Geometry: final body of the model. Coordinates: model frame, mm. A direction names the side the tool comes from. Give positions to 0.01 mm unless a question says otherwise; leave off trailing zeros. Loops run counter-clockwise (first coordinate to the right, second up) from the corner with the lowest first, then second, coordinate; pieces in that order, holes last. Notation, with made-up numbers: (12, 47) -> (56, 47) arc R31 cw to (56, 77) -> close; hole circle Ø11 at (-38.5, 65.5). An arc over 180 degrees is marked (long way). Answer in a Markdown table with one row per item. Add a question column.
1) Section query A-A (x = 40). Return the cut outline in (y, z).
2) Section query D-D (x = 105). Return the cut outline in (y, z).
3) Access query for faces 1 (the flat face through (25, 10, 5)), 2 (the flat face through (40, 6.8, 56)), 3 (the cylindrical face through (-40.43, 9.44, 49.23)). Directions: +Z, -Z, +X, -X, +Y, -Y. A direction counts if a zero-diameter tool reaches every point of the face in a straight line with its end or side. Return the directions, or none.
4) Section query C-C (z = -45). Return the cut outline in (x, y).
5) Line query: line 1 (X direction, y = 10.25, z = -45); line 2 (Z direction, x = -105, y = 10); line 3 (X direction, y = 10.6, z = 52.5). Output: solid intervals per line, ascending. Write a range as from..to.
6) First-contact query: P1, Ø3.5, axis at x = -103, z = -46, coming from the -Y side; P2, Ø3, axis at x = -24, z = 5, coming from the +Y side; P3, Ø6, axis at x = -105, z = 45, coming from the +Y side. Flat tips, straight axial feed; report the tip coordinate or a pass-through.
7) Draft query along Z for faces 4 (the cylindrical face through (110.495, 3.352, 44.758)), 5 (the flat face through (-2, 6, 72.5)), 6 (the flat face through (-2, 12, -1)). Return one class per face: +Z half, -Z half, draft (parallel to the pull), parting line (faces both ways), or undercut.
8) Section query B-B (z = -20). Return the cut outline in (x, y), plus the area to 3 significant figures.
```python
from build123d import *

# Parameters (mm, degrees)
SKETCH_1_W                   = 250
SKETCH_1_H                   = 145
EXTRUDE_1_DEPTH              = 12
CHAMFER_1_SIZE               = 2
SKETCH_2_R                   = 18
CUT_EXTRUDE_1_DEPTH          = 146.000862066
HOLE_WIZARD_M4_1_D           = 3.3
HOLE_WIZARD_M6_1_D           = 6.6
HOLE_WIZARD_M6_1_CBORE_D     = 11
HOLE_WIZARD_M6_1_CBORE_DEPTH = 6.8
SKETCH_11_R                  = 5
CUT_EXTRUDE_2_DEPTH          = 2


with BuildPart() as part:
    # 草图1 → 凸台-拉伸1 (new body)
    with BuildSketch(Plane(origin=(0, 0, 0), x_dir=(1, 0, 0), z_dir=(0, 1, 0))):
        Rectangle(SKETCH_1_W, SKETCH_1_H)
    extrude(amount=EXTRUDE_1_DEPTH)

    # 倒角1
    chamfer_1_edges = [part.edges().sort_by_distance(p)[0] for p in [
        (125, 6, 72.5),
        (-125, 6, 72.5),
        (-125, 6, -72.5),
        (125, 6, -72.5),
    ]]
    chamfer(chamfer_1_edges, length=CHAMFER_1_SIZE)

    # 草图2 → 切除-拉伸1 (cut, through all)
    with BuildSketch(Plane(origin=(0, 12, 0), x_dir=(1, 0, 0), z_dir=(0, 1, 0))):
        with Locations(Location((0, 20, 0), (0, 0, 270))):
            Circle(SKETCH_2_R)
    extrude(amount=-CUT_EXTRUDE_1_DEPTH, mode=Mode.SUBTRACT)

    # M4 螺纹孔1 (through all)
    with Locations(Plane(origin=(0, 0, 0), x_dir=(-1, 0, 0), z_dir=(0, -1, 0))):
        with Locations((15.556349186, 35.556349186), (-15.556349186, 35.556349186), (-15.556349186, 4.443650814), (15.556349186, 4.443650814)):
            Hole(HOLE_WIZARD_M4_1_D / 2)

    # M6 六角圆柱头螺钉的柱形沉头孔1 (through all)
    with Locations(Plane(origin=(0, 0, 0), x_dir=(-1, 0, 0), z_dir=(0, -1, 0))):
        with Locations((-40, -52.5), (-105, 45), (-105, -45), (105, 45), (105, -45), (40, -52.5)):
            CounterBoreHole(HOLE_WIZARD_M6_1_D / 2, HOLE_WIZARD_M6_1_CBORE_D / 2, HOLE_WIZARD_M6_1_CBORE_DEPTH)

    # 草图11 → 切除-拉伸2 (cut)
    with BuildSketch(Plane(origin=(0, 12, 0), x_dir=(1, 0, 0), z_dir=(0, 1, 0))):
        with Locations(Location((24.748737342, -4.748737342, 0), (0, 0, 270))):
            Circle(SKETCH_11_R)
        with Locations(Location((-24.748737342, -4.748737342, 0), (0, 0, 270))):
            Circle(SKETCH_11_R)
        with Locations(Location((-24.748737342, 44.748737342, 0), (0, 0, 270))):
            Circle(SKETCH_11_R)
        with Locations(Location((24.748737342, 44.748737342, 0), (0, 0, 270))):
            Circle(SKETCH_11_R)
    extrude(amount=-CUT_EXTRUDE_2_DEPTH, mode=Mode.SUBTRACT)


solid = part.part
```
Evaluation:
| question | item | result |
|---|---|---|
| 1 | outline | (0, -72.5) -> (12, -72.5) -> (12, 49.2) -> (6.8, 49.2) -> (6.8, 47) -> (0, 47) -> close; (0, 58) -> (6.8, 58) -> (6.8, 55.8) -> (12, 55.8) -> (12, 72.5) -> (0, 72.5) -> close |
| 2 | outline | (0, -72.5) -> (12, -72.5) -> (12, -48.3) -> (6.8, -48.3) -> (6.8, -50.5) -> (0, -50.5) -> close; (0, -39.5) -> (6.8, -39.5) -> (6.8, -41.7) -> (12, -41.7) -> (12, 41.7) -> (6.8, 41.7) -> (6.8, 39.5) -> (0, 39.5) -> close; (0, 50.5) -> (6.8, 50.5) -> (6.8, 48.3) -> (12, 48.3) -> (12, 72.5) -> (0, 72.5) -> close |
| 3 | face 1 | +Y |
| 3 | face 2 | -Y |
| 3 | face 3 | +Y, -Y |
| 4 | outline | (-125, 0) -> (-110.5, 0) -> (-110.5, 6.8) -> (-108.3, 6.8) -> (-108.3, 12) -> (-125, 12) -> close; (-101.7, 6.8) -> (-99.5, 6.8) -> (-99.5, 0) -> (99.5, 0) -> (99.5, 6.8) -> (101.7, 6.8) -> (101.7, 12) -> (29.74, 12) -> (29.74, 10) -> (19.76, 10) -> (19.76, 12) -> (-19.76, 12) -> (-19.76, 10) -> (-29.74, 10) -> (-29.74, 12) -> (-101.7, 12) -> close; (108.3, 6.8) -> (110.5, 6.8) -> (110.5, 0) -> (125, 0) -> (125, 12) -> (108.3, 12) -> close |
| 5 | line 1 | -125..-108.3, -101.7..-29.74, -19.76..19.76, 29.74..101.7, 108.3..125 |
| 5 | line 2 | -72.5..-48.3, -41.7..41.7, 48.3..72.5 |
| 5 | line 3 | -125..-43.3, -36.7..36.7, 43.3..125 |
| 6 | P1 | y = 6.8 |
| 6 | P2 | y = 10 |
| 6 | P3 | through |
| 7 | face 4 | undercut |
| 7 | face 5 | +Z half |
| 7 | face 6 | draft |
| 8 | outline | (-125, 0) -> (-18, 0) -> (-18, 12) -> (-125, 12) -> close; (18, 0) -> (125, 0) -> (125, 12) -> (18, 12) -> close |
| 8 | area | 2,570 mm² |
